Could you check a few things on this drawing? It's one solid part, dimensions in mm from its lowest x, y, z. A direction names the side the tool comes from. Coordinates: 2 decimals unless noted, no trailing zeros. Order: outer loops, then holes, each group sorted by start corner. A loop starts at its lowest first (then second) coordinate and runs counter-clockwise, first axis right, second up. Notation, with made-up numbers: M 21,40 L 71,40 A17 cw 71,73 Z; hole C 53,87 d8. An arc over 180 degrees is marked long. One line per question, with ' | ' between items. Start each with the question number.
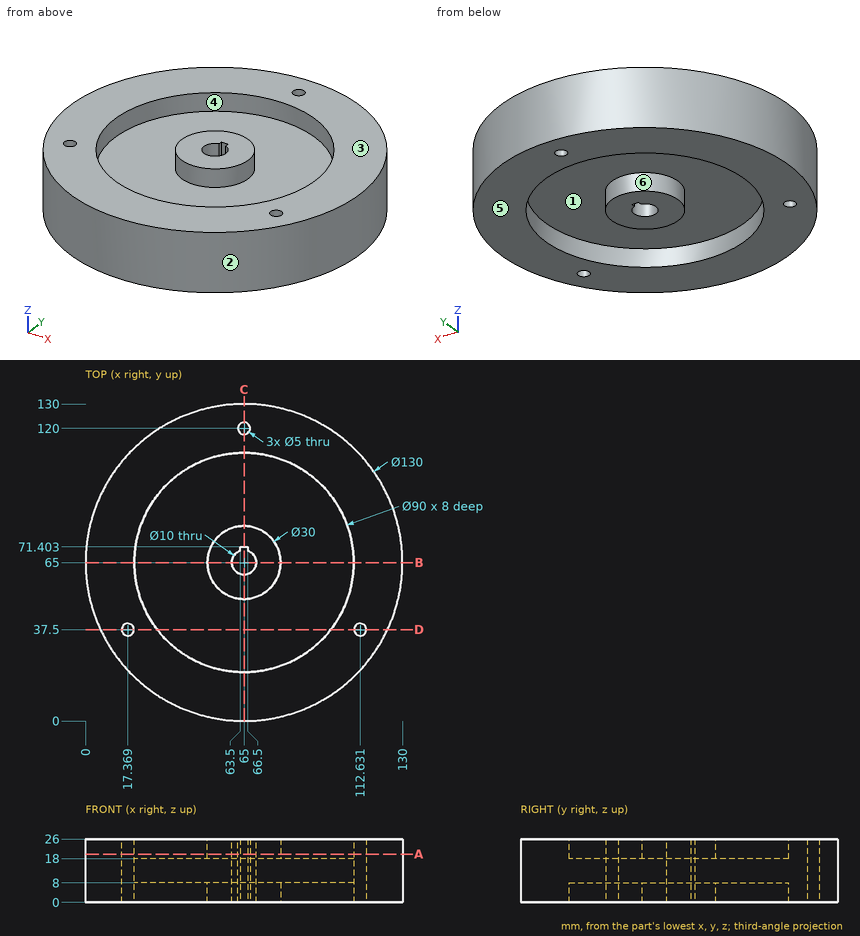
1. Which directions (+Z, -Z, +X, -X, +Y, -Y) give clear straight access to the entire face, cutting with the end or side of a thin tool? Please do the marked faces 4, 5 and 6.
2. Imagine slicing it at D-D (y = 37.5). List the corners of the cut face in (x, z) for me, then the cut area to 3 significant figures.
3. We'd pull the mould along X, two halves only. Please class the marked faces 1, 2 and 3: released by +X, released by -X, zero draft, split by the parting line, or undercut.
4. Imagine slicing it at B-B (y = 65). List the corners of the cut face in (x, z) for me.
5. Imagine slicing it at C-C (x = 65). List the corners of the cut face in (y, z) for me.
6. I need wall thicknesses on line 1 (Y direction, x = 65, z = 17.25); line 2 (Y direction, x = 65, z = 4); line 3 (X direction, y = 37.5, z = 12) (1 decimal). Which ranges of each line are inside material? Lowest first, please.
7. Imagine slicing it at A-A (z = 19.75). List the corners of the cut face in (x, y) for me.
8. Will these pins go through, and if not, where does the flat tip stop? pin 1 (1.5 mm diameter, centred on x = 25.5, y = 60.5, fed in from -Z); pin 2 (1 mm diameter, centred on y = 79, z = 13.5, fed in from -X); pin 3 (1 mm diameter, centred on x = 108, z = 23, fed in from -Y).
Entries:
1) face 4: +Z | face 5: -Z, +X, -X, +Y, -Y | face 6: -Z
2) outline: M 6.1,0 L 14.87,0 L 14.87,26 L 6.1,26 Z; M 19.87,0 L 29.38,0 L 29.38,8 L 100.62,8 L 100.62,0 L 110.13,0 L 110.13,26 L 100.62,26 L 100.62,18 L 29.38,18 L 29.38,26 L 19.87,26 Z; M 115.13,0 L 123.9,0 L 123.9,26 L 115.13,26 Z | area: 1,660 mm²
3) face 1: undercut | face 2: split by the parting line | face 3: zero draft
4) outline: M 0,0 L 20,0 L 20,8 L 50,8 L 50,0 L 60,0 L 60,26 L 50,26 L 50,18 L 20,18 L 20,26 L 0,26 Z; M 70,0 L 80,0 L 80,8 L 110,8 L 110,0 L 130,0 L 130,26 L 110,26 L 110,18 L 80,18 L 80,26 L 70,26 Z
5) outline: M 0,0 L 20,0 L 20,8 L 50,8 L 50,0 L 60,0 L 60,26 L 50,26 L 50,18 L 20,18 L 20,26 L 0,26 Z; M 71.4,0 L 80,0 L 80,8 L 110,8 L 110,0 L 117.5,0 L 117.5,26 L 110,26 L 110,18 L 80,18 L 80,26 L 71.4,26 Z; M 122.5,0 L 130,0 L 130,26 L 122.5,26 Z
6) line 1: 0 to 60, 71.4 to 117.5, 122.5 to 130 | line 2: 0 to 20, 50 to 60, 71.4 to 80, 110 to 117.5, 122.5 to 130 | line 3: 6.1 to 14.9, 19.9 to 110.1, 115.1 to 123.9
7) outline: C 65,65 d130; C 65,65 d30; hole C 17.37,37.5 d5; hole C 65,65 d90; hole C 65,120 d5; hole M 63.5,69.77 A5 ccw long 66.5,69.77 L 66.5,71.4 L 63.5,71.4 Z; hole C 112.63,37.5 d5
8) pin 1: z = 8 | pin 2: x = 1.42 | pin 3: y = 15.82
